from build123d import *

# Parameters (mm, degrees)
SKETCH1_R           = 1.5
BOSS_EXTRUDE1_DEPTH = 3


with BuildPart() as part:
    # Sketch1 → Boss-Extrude1 (new body)
    with BuildSketch(Plane.XY):
        with BuildLine():
            Line((-69.019918417, -6.227312299), (-59.101906393, -6.196290568))
            Line((-59.101906393, -6.196290568), (-48.926464715, -6.227677735))
            Line((-48.926464715, -6.227677735), (-9.807058311, -4.032732904))
            Line((-9.807058311, -4.032732904), (9.82e-05, -4.000021922))
            Line((9.82e-05, -4.000021922), (10.060192173, -4.033082606))
            Line((10.060192173, -4.033082606), (57.060189179, -4.206563863))
            Line((57.060189179, -4.206563863), (67.179803064, -3.520371058))
            Line((67.179803064, -3.520371058), (77.15689228, -2.843842595))
            ThreePointArc((77.15689228, -2.843842595), (80.877116582, 1.417604476), (76.61566951, 5.137828778))
            Line((76.61566951, 5.137828778), (66.638580293, 4.461300315))
            Line((66.638580293, 4.461300315), (56.804015745, 3.794436193))
            Line((56.804015745, 3.794436193), (10.088101644, 3.966868874))
            Line((10.088101644, 3.966868874), (-9.82e-05, 4.000021922))
            Line((-9.82e-05, 4.000021922), (-10.044647872, 3.966519135))
            Line((-10.044647872, 3.966519135), (-49.138394535, 1.773014043))
            Line((-49.138394535, 1.773014043), (-59.102079262, 1.803748024))
            Line((-59.102079262, 1.803748024), (-69.044940833, 1.772648568))
            ThreePointArc((-69.044940833, 1.772648568), (-73.032410059, -2.239843074), (-69.019918417, -6.227312299))
        make_face()
        with Locations((-69.032429625, -2.227331865)):
            Circle(SKETCH1_R, mode=Mode.SUBTRACT)
        with Locations((-59.101992828, -2.196271272)):
            Circle(SKETCH1_R, mode=Mode.SUBTRACT)
        with Locations((-49.032429625, -2.227331846)):
            Circle(SKETCH1_R, mode=Mode.SUBTRACT)
        with Locations((-9.925853092, -0.033106885)):
            Circle(SKETCH1_R, mode=Mode.SUBTRACT)
        Circle(SKETCH1_R, mode=Mode.SUBTRACT)
        with Locations((10.074146909, -0.033106866)):
            Circle(SKETCH1_R, mode=Mode.SUBTRACT)
        with Locations((56.932102462, -0.206063835)):
            Circle(SKETCH1_R, mode=Mode.SUBTRACT)
        with Locations((66.909191678, 0.470464628)):
            Circle(SKETCH1_R, mode=Mode.SUBTRACT)
        with Locations((76.886280895, 1.146993091)):
            Circle(SKETCH1_R, mode=Mode.SUBTRACT)
    extrude(amount=BOSS_EXTRUDE1_DEPTH)


solid = part.part
The model under review builds one solid part; all positions refer to its coordinate system, in mm. Give positions to 0.01 mm unless a question says otherwise; leave off trailing zeros. Write each loop counter-clockwise with the first axis right and the second up, starting at its lowest first coordinate (ties: lowest second). Pieces come first, ordered by that corner, then holes.
1. Add section B-B, the plane x = -29. Write out the cut boundary in (y, z).
2. For P1, Ø2, axis at x = -51.5, y = -1, coming from the -Z side; P2, Ø1.5, axis at y = 1, z = 1.5, coming from the -X side, all flat-tipped, find the tip position at first contact; note any pin that passes through.
3. Draft analysis for pull direction Y (two halves, no side actions). For faces 1 (the cylindrical face through (80.882, 1.33, 1.479)), 2 (the cylindrical face through (-57.67, -1.75, 1.48)), 3 (the cylindrical face through (55.742, -1.119, 1.479)), 4 (the flat face through (3, 0, 0)), state which applies: +Y half, -Y half, draft (parallel to the pull), parting line (faces both ways), or undercut.
4. Add section C-C, the plane x = 64. Write out the cut boundary in (y, z), plus the area to 3 significant figures.
5. Add section A-A, the plane z = 2.3. Count the separate pieces of the cut face and the enclosed holes in it, plus the area to 3 significant figures.
6. Wall thickness on L1, parallel to X at y = -1.75, z = 1.35; L2, parallel to Y at x = 58, z = 0.7; L3, parallel to Y at x = -2, z = 2.25: over which ranges is each line inside the solid? List them lowest first.
Worked answers:
1. outline: (-5.11, 0) - (2.9, 0) - (2.9, 3) - (-5.11, 3) - close
2. P1: stops at z = 0
2. P2: stops at x = -72.17
3. face 1: parting line
3. face 2: undercut
3. face 3: undercut
3. face 4: draft
4. outline: (-3.74, 0) - (4.28, 0) - (4.28, 3) - (-3.74, 3) - close
4. area: 24.1 mm2
5. separate pieces: 1
5. enclosed holes: 9
5. area: 1,150 mm2
6. L1: x = -73 to -70.45, -67.61 to -60.53, -57.67 to -50.45, -47.61 to 79.64
6. L2: y = -4.14 to -1.26, 0.85 to 3.88
6. L3: y = -4.01 to 3.99
